from build123d import *

# Parameters (mm, degrees)
EXTRUDE_972_DEPTH      = 0.75
EXTRUDE_972_DEPTH_BACK = 0.75
SKETCH_1_R             = 1.5


with BuildPart() as part:
    # 草图1 → Extrude 972 (new, two sides: drawn at the far end of the back side and taken through both)
    with BuildSketch(Plane.XY.offset(-EXTRUDE_972_DEPTH_BACK)):
        with BuildLine():
            Line((-1.5, -21.945712116), (-1.5, -28.709060435))
            ThreePointArc((-1.5, -28.709060435), (-5.322611287, -28.229989049), (-9.040763088, -27.22141896))
            ThreePointArc((-9.040763088, -27.22141896), (-9.343684575, -27.01404373), (-9.5, -26.68188202))
            Line((-9.5, -26.68188202), (-10.150143719, -22.994733766))
            ThreePointArc((-10.150143719, -22.994733766), (-10.42496916, -22.358396436), (-10.956546386, -21.91355953))
            ThreePointArc((-10.956546386, -21.91355953), (0, 24.5), (10.956546386, -21.91355953))
            ThreePointArc((10.956546386, -21.91355953), (10.42496916, -22.358396436), (10.150143719, -22.994733766))
            Line((10.150143719, -22.994733766), (9.5, -26.68188202))
            ThreePointArc((9.5, -26.68188202), (9.343684575, -27.01404373), (9.040763088, -27.22141896))
            ThreePointArc((9.040763088, -27.22141896), (5.322611287, -28.229989049), (1.5, -28.709060435))
            Line((1.5, -28.709060435), (1.5, -21.945712116))
            ThreePointArc((1.5, -21.945712116), (0, 19.5), (-1.5, -21.945712116))
        make_face()
        with Locations((-5.5, -24.714015002)):
            Circle(SKETCH_1_R, mode=Mode.SUBTRACT)
        with Locations(Location((5.5, -24.714015002, 0), (0, 0, 180))):
            Circle(SKETCH_1_R, mode=Mode.SUBTRACT)
    extrude(amount=EXTRUDE_972_DEPTH + EXTRUDE_972_DEPTH_BACK)


solid = part.part
Design review of the part built by this model. Coordinates are the model's own, in mm. Coordinates: 2 decimals unless noted, no trailing zeros. Write each loop counter-clockwise with the first axis right and the second up, starting at its lowest first coordinate (ties: lowest second). Pieces come first, ordered by that corner, then holes. Notation, with made-up numbers: (-8.75, 3) - (39.25, 3) arc R18 ccw to (39.25, 31) - close; hole circle Ø8 at (25, 22.25). An arc over 180 degrees is marked (long way). Use one line per item in the form item = value.
Q1. The part is to be moulded in two halves that separate along X. For faces 1 (the flat face through (1.5, -25, 0)), 2 (the flat face through (-1.5, -25, 0)), 3 (the cylindrical face through (-0.918, 24.483, -0.01)), 4 (the cylindrical face through (5.38, -28.22, -0.01)), say which applies: +X half, -X half, draft (parallel to the pull), parting line (faces both ways), or undercut.
Taken from the geometry:
face_1 = undercut
face_2 = undercut
face_3 = parting line
face_4 = +X half
Q2. Consider section D-D (x = 5.5). Write out the cut boundary in (y, z).
Taken from the geometry:
outline = (-28.19, -0.75) - (-26.21, -0.75) - (-26.21, 0.75) - (-28.19, 0.75) - close; (-23.21, -0.75) - (-21.26, -0.75) - (-21.26, 0.75) - (-23.21, 0.75) - close; (18.76, -0.75) - (23.87, -0.75) - (23.87, 0.75) - (18.76, 0.75) - close
Q3. Consider section A-A (z = -0.3). Write out the cut boundary in (x, y), plus the area to 3 significant figures.
Taken from the geometry:
outline = (-10.96, -21.91) arc R1.5 cw to (-10.15, -22.99) - (-9.5, -26.68) arc R0.7 ccw to (-9.04, -27.22) arc R27.5 ccw to (-1.5, -28.71) - (-1.5, -21.95) arc R20.75 cw (long way) to (1.5, -21.95) - (1.5, -28.71) arc R27.5 ccw to (9.04, -27.22) arc R0.7 ccw to (9.5, -26.68) - (10.15, -22.99) arc R1.5 cw to (10.96, -21.91) arc R24.5 ccw (long way) to start; hole circle Ø3 at (-5.5, -24.71); hole circle Ø3 at (5.5, -24.71)
area = 584 mm^2
Q4. Consider section B-B (y = 14.5). Write out the cut boundary in (x, z), plus the area to 3 significant figures.
Taken from the geometry:
outline = (-19.75, -0.75) - (-13.51, -0.75) - (-13.51, 0.75) - (-19.75, 0.75) - close; (13.51, -0.75) - (19.75, -0.75) - (19.75, 0.75) - (13.51, 0.75) - close
area = 18.7 mm^2
Q5. Consider section C-C (x = -17). Write out the cut boundary in (y, z), plus the area to 3 significant figures.
Taken from the geometry:
outline = (-17.64, -0.75) - (-13.15, -0.75) - (-13.15, 0.75) - (-17.64, 0.75) - close; (10.65, -0.75) - (17.64, -0.75) - (17.64, 0.75) - (10.65, 0.75) - close
area = 17.2 mm^2
Q6. For probe 1 along Y at (x, z) = (-5, -0.4); probe 2 along Y at (x, z) = (5.5, -0.1); probe 3 along X at (y, z) = (9, -0.6), list the stretches that pass through material, from the lowest coordinate up.
Taken from the geometry:
probe_1 = -28.29 to -26.13, -23.3 to -21.39, 18.89 to 23.98
probe_2 = -28.19 to -26.21, -23.21 to -21.26, 18.76 to 23.87
probe_3 = -22.79 to -18.04, 18.04 to 22.79
Q7. Insertion check: pin 1 Ø4 at (x, y) = (5.5, -24.71) entering from +Z. The pin has a flat end and moves straight along its axis. Give the tip position at first contact, or say it passes through.
Taken from the geometry:
pin_1 = 0.75
